Input: dimensioned drawing with shaded views. Units: mm. Origin: part minimum x, y, z. A direction names the side the tool comes from. Round coordinates to 2 decimals unless told otherwise and drop trailing zeros. Order: outer loops, then holes, each group sorted by start corner. A loop starts at its lowest first (then second) coordinate and runs counter-clockwise, first axis right, second up. Notation, with made-up numbers: M 77.25,53 L 81.25,53 A4 ccw 81.25,59 Z; hole C 16,-30.5 d9. An arc over 180 degrees is marked long. Put each result on its own line as item: value. Start each with the question number.
1) Section B-B, the plane y = 15. Return loops of the section in (x, z).
2) Material intervals for probe 1 along Z at (x, y) = (5.5, 6.25); probe 2 along X at (y, z) = (3, 4), sorted ascending. Write a range as [from, to].
3) Draft query along Y for the marked faces 1, 2 and 3. Return one class per face: pulls with the +Y half, pulls with the -Y half, needs draft (parallel to the pull), parting line crosses it, or undercut.
4) Section C-C, the plane y = 7.25. Return loops of the section in (x, z), then the cut area to 3 significant figures.
5) Access query for the marked faces 4 and 5. Directions: +Z, -Z, +X, -X, +Y, -Y. A direction counts if a zero-diameter tool reaches every point of the face in a straight line with its end or side. Return the directions, or none.
6) Section D-D, the plane z = 1.5. Return loops of the section in (x, y), then the cut area to 3 significant figures.
7) Section A-A, the plane x = 12.5. Return loops of the section in (y, z).
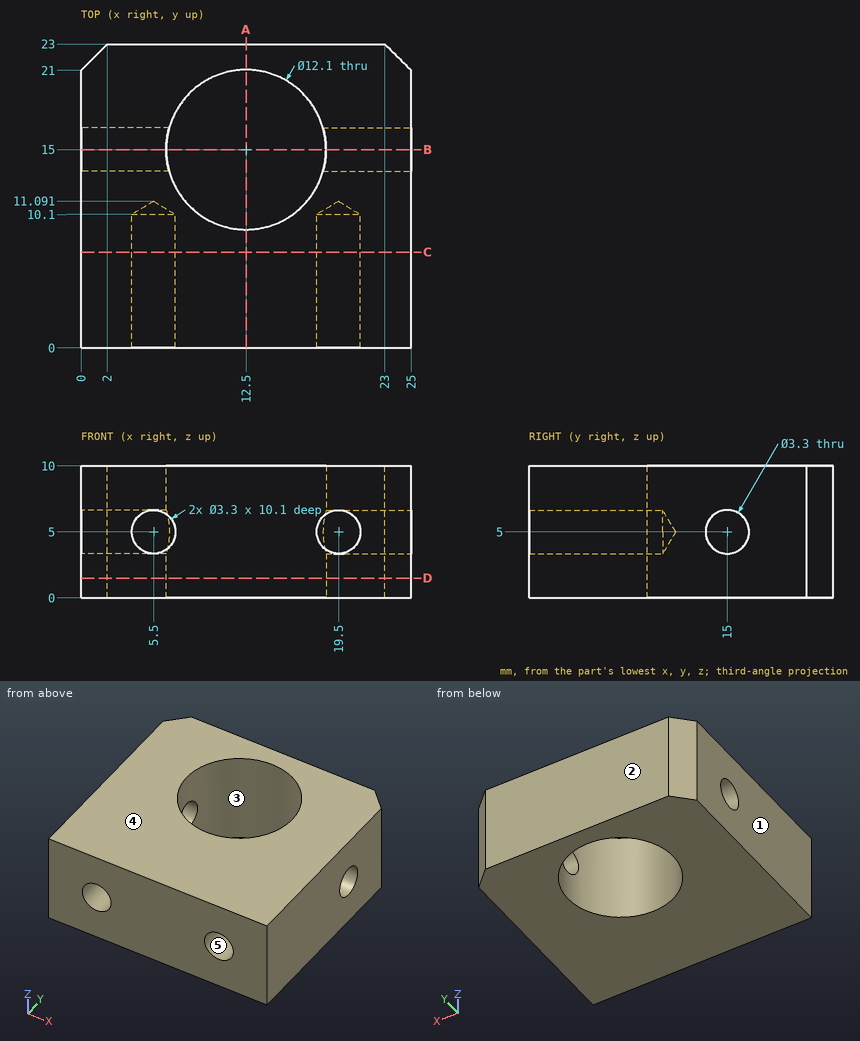
Result sheet:
1. outline: M 0,0 L 6.45,0 L 6.45,3.35 L 0,3.35 Z; M 0,6.65 L 6.45,6.65 L 6.45,10 L 0,10 Z; M 18.55,0 L 25,0 L 25,3.35 L 18.55,3.35 Z; M 18.55,6.65 L 25,6.65 L 25,10 L 18.55,10 Z
2. probe 1: z = [0, 3.35], [6.65, 10]
2. probe 2: x = [0, 4.19], [6.81, 18.19], [20.81, 25]
3. face 1: needs draft
3. face 2: pulls with the +Y half
3. face 3: undercut
4. outline: M 0,0 L 25,0 L 25,10 L 0,10 Z; hole C 5.5,5 d3.3; hole C 19.5,5 d3.3
4. area: 233 mm2
5. face 4: +Z, +X, -X, +Y, -Y
5. face 5: -Y
6. outline: M 0,0 L 25,0 L 25,21 L 23,23 L 2,23 L 0,21 Z; hole C 12.5,15 d12.1
6. area: 456 mm2
7. outline: M 0,0 L 8.95,0 L 8.95,10 L 0,10 Z; M 21.05,0 L 23,0 L 23,10 L 21.05,10 Z
